from build123d import *

# Parameters (mm, degrees)
SKETCH1_W           = 10
SKETCH1_H           = 30
BOSS_EXTRUDE1_START = 30
BOSS_EXTRUDE1_DEPTH = 30
BOSS_EXTRUDE2_START = 360
SKETCH3_R           = 10
BOSS_EXTRUDE2_DEPTH = 360


with BuildPart() as part:
    # Sketch1 → Revolve1 (revolve)
    with BuildSketch(Plane(origin=(0, 0, 0), x_dir=(1, 0, 0), z_dir=(0, 1, 0))):
        with Locations((5, -30)):
            Rectangle(SKETCH1_W, SKETCH1_H)
    revolve(axis=Axis((0, 0, 15), (0, 0, 1)))

    # Sketch2 → Boss-Extrude1 (add)
    with BuildSketch(Plane(origin=(0, 0, 15), x_dir=(-1, 0, 0), z_dir=(0, 0, -1)).offset(BOSS_EXTRUDE1_START)):
        with BuildLine():
            Line((-5, 8.660254038), (-6.5, 11.258330249))
            ThreePointArc((-6.5, 11.258330249), (11.258330249, -6.5), (-13, 0))
            Line((-13, 0), (-13, 57))
            Line((-13, 57), (-200, 57))
            ThreePointArc((-200, 57), (-202.5, 47.669872981), (-195.669872981, 54.5))
            Line((-195.669872981, 54.5), (-193.07179677, 56))
            ThreePointArc((-193.07179677, 56), (-204, 45.07179677), (-200, 60))
            Line((-200, 60), (-10, 60))
            Line((-10, 60), (-10, 0))
            ThreePointArc((-10, 0), (-8.660254038, 5), (-5, 8.660254038))
        make_face()
    extrude(amount=-BOSS_EXTRUDE1_DEPTH)

    # Sketch3 → Boss-Extrude2 (add)
    with BuildSketch(Plane(origin=(0, 0, -15), x_dir=(-1, 0, 0), z_dir=(0, 0, -1)).offset(BOSS_EXTRUDE2_START)):
        with Locations(Location((0, 0, 0), (0, 0, 180))):
            Circle(SKETCH3_R)
    extrude(amount=-BOSS_EXTRUDE2_DEPTH)


solid = part.part
Source: CAD feature listing. Evaluate the final solid. Frame: model axes, mm. A direction names the side the tool comes from. Coordinates: 2 decimals unless noted, no trailing zeros. Loops run counter-clockwise (first coordinate to the right, second up) from the corner with the lowest first, then second, coordinate; pieces in that order, holes last. Notation, with made-up numbers: (83, -14.75) -> (99, -14.75) arc R35 cw to (99, 24.25) -> close; hole circle Ø7 at (43, 35). An arc over 180 degrees is marked (long way). Answer in a Markdown table with one row per item. Add a question column.
Q1. Reachability of faces 3 (the face through (13, 28, 0)), 4 (the face through (0, 0, -375)) from +Z, -Z, +X, -X, +Y, -Y: full face, straight path, thin tool, end or side. Return the list, or none.
Q2. Pull-direction query (X, two-part tool) for faces 1 (the face through (203.74, 44.93, -0.21)), 2 (the face through (89, 59, -15)); classes: pulls with the +X half, pulls with the -X half, needs draft (parallel to the pull), parting line crosses it, or undercut.
Q3. Section D-D on z = -233. Return the cut outline in (x, y), and give its area (3 significant figures).
Q4. Section C-C on x = 63. Return the cut outline in (y, z).
Q5. Section A-A on x = 0. Return the cut outline in (y, z), and give its area (3 significant figures).
Q6. Ray query, line 1 along X through (y, z) = (52, -7.25); line 2 along Y through (x, z) = (38, -13.5); line 3 along X through (y, z) = (54, -2.5). Return the intervals inside material, ascending.
Q7. Contact query for flat-ended pins moving along their axis: pin 1 Ø13 at (x, y) = (200, 52) entering from -Z; pin 2 Ø12 at (y, z) = (29, -14) entering from +X; pin 3 Ø15 at (x, z) = (88, -6.5) entering from -Y. Output: stop coordinate, or through.
Q8. Section B-B on z = 5. Return the cut outline in (x, y), and give its area (3 significant figures).
Computed values:
| question | item | result |
|---|---|---|
| 1 | face 3 | +Z, -Z, -Y |
| 1 | face 4 | -Z, +X, -X, +Y, -Y |
| 2 | face 1 | undercut |
| 2 | face 2 | needs draft |
| 3 | outline | circle Ø20 at (0, 0) |
| 3 | area | 314 mm^2 |
| 4 | outline | (57, -15) -> (60, -15) -> (60, 15) -> (57, 15) -> close |
| 5 | outline | (-13, -15) -> (-10, -15) -> (-10, -375) -> (10, -375) -> (10, -15) -> (13, -15) -> (13, 15) -> (10, 15) -> (10, 45) -> (-10, 45) -> (-10, 15) -> (-13, 15) -> close |
| 5 | area | 8,580 mm^2 |
| 6 | line 1 | x = 10 to 13, 192 to 195, 205 to 208 |
| 6 | line 2 | y = 57 to 60 |
| 6 | line 3 | x = 10 to 13, 192.25 to 195.42, 204.58 to 207.75 |
| 7 | pin 1 | stops at z = -15 |
| 7 | pin 2 | stops at x = 13 |
| 7 | pin 3 | stops at y = 57 |
| 8 | outline | (5, 8.66) -> (6.5, 11.26) arc R13 ccw (long way) to (13, 0) -> (13, 57) -> (200, 57) arc R5 cw (long way) to (195.67, 54.5) -> (193.07, 56) arc R8 ccw (long way) to (200, 60) -> (10, 60) -> (10, 0) arc R10 ccw to start |
| 8 | area | 1,340 mm^2 |
